Geometry: final body of the model. Coordinates: model frame, mm. A direction names the side the tool comes from. Round coordinates to 2 decimals unless told otherwise and drop trailing zeros. Loops run counter-clockwise (first coordinate to the right, second up) from the corner with the lowest first, then second, coordinate; pieces in that order, holes last. Notation, with made-up numbers: (54.25, 87) -> (67.25, 87) arc R21 ccw to (67.25, 122) -> close; hole circle Ø5 at (-4.5, 36). An arc over 180 degrees is marked (long way). Answer in a Markdown table with one row per item.
```python
from build123d import *

# Parameters (mm, degrees)
SKETCH1_R           = 9
BOSS_EXTRUDE1_DEPTH = 63
SKETCH2_R           = 10
BOSS_EXTRUDE2_DEPTH = 48
SKETCH3_R           = 6
CUT_EXTRUDE1_DEPTH  = 65.567793829
SKETCH4_W           = 1.5
SKETCH4_H           = 27.68
CIRPATTERN1_COUNT   = 4
CHAMFER1_SIZE       = 0.5


with BuildPart() as part:
    # Sketch1 → Boss-Extrude1 (new body)
    with BuildSketch(Plane.XY):
        Circle(SKETCH1_R)
    extrude(amount=BOSS_EXTRUDE1_DEPTH)

    # Sketch2 → Boss-Extrude2 (add)
    with BuildSketch(Plane(origin=(0, 0, 0), x_dir=(-1, 0, 0), z_dir=(0, 0, -1))):
        Circle(SKETCH2_R)
    extrude(amount=-BOSS_EXTRUDE2_DEPTH)

    # Sketch3 → Cut-Extrude1 (cut, through all)
    with BuildSketch(Plane(origin=(0, 0, 0), x_dir=(-1, 0, 0), z_dir=(0, 0, -1))):
        Circle(SKETCH3_R)
    extrude(amount=-CUT_EXTRUDE1_DEPTH, mode=Mode.SUBTRACT)

    # Sketch4 → Cut-Revolve1 (revolve, cut)
    with BuildSketch(Plane(origin=(0, 0, 0), x_dir=(0, 0, -1), z_dir=(1, 0, 0)), mode=Mode.PRIVATE) as cut_revolve1_sk:
        with Locations((-25.75, 0.585439351)):
            Rectangle(SKETCH4_W, SKETCH4_H)
    cut_revolve1 = revolve(cut_revolve1_sk.sketch.rotate(Axis((0, 14.425439351, 26.5), (0, -1, 0)), 180), axis=Axis((0, 14.425439351, 26.5), (0, -1, 0)), mode=Mode.SUBTRACT)

    # CirPattern1: Cut-Revolve1 ×4 about axis
    cirpattern1_axis = Axis((0, 0, 48), (0, 0, -1))
    for i in range(1, CIRPATTERN1_COUNT):
        add(cut_revolve1.rotate(cirpattern1_axis, i * 360 / CIRPATTERN1_COUNT), mode=Mode.SUBTRACT)

    # Chamfer1
    chamfer1_edges = [part.edges().sort_by_distance(p)[0] for p in [
        (6, 0, 63),
    ]]
    chamfer(chamfer1_edges, length=CHAMFER1_SIZE)


solid = part.part
```
Item 1: First-contact query: P1, Ø1.5, axis at y = -5.5, z = 55.5, coming from the +X side; P2, Ø5, axis at x = -1, z = 49.5, coming from the +Y side; P3, Ø1.8, axis at y = 0, z = 26.5, coming from the -X side; P4, Ø2, axis at x = -1.5, z = 55, coming from the -Y side. Flat tips, straight axial feed; report the tip coordinate or a pass-through.
Ans:
| item | result |
|---|---|
| P1 | x = 7.64 |
| P2 | y = 10 |
| P3 | through |
| P4 | y = -8.99 |
Item 2: Section query A-A, the plane y = 0. Output: boundary loops of the cut face in (x, z), and give its area (3 significant figures).
Ans:
| item | result |
|---|---|
| outline | (-10, 0) -> (-6, 0) -> (-6, 25) -> (-10, 25) -> close; (-10, 28) -> (-6, 28) -> (-6, 62.5) -> (-6.5, 63) -> (-9, 63) -> (-9, 48) -> (-10, 48) -> close; (6, 0) -> (10, 0) -> (10, 25) -> (6, 25) -> close; (6, 28) -> (10, 28) -> (10, 48) -> (9, 48) -> (9, 63) -> (6.5, 63) -> (6, 62.5) -> close |
| area | 450 mm2 |
Item 3: Section query C-C, the plane z = 26.5. Output: boundary loops of the cut face in (x, y), and give its area (3 significant figures).
Ans:
| item | result |
|---|---|
| outline | (-9.89, -1.5) arc R10 ccw to (-1.5, -9.89) -> (-1.5, -5.81) arc R6 cw to (-5.81, -1.5) -> close; (-9.89, 1.5) -> (-5.81, 1.5) arc R6 cw to (-1.5, 5.81) -> (-1.5, 9.89) arc R10 ccw to start; (1.5, -9.89) arc R10 ccw to (9.89, -1.5) -> (5.81, -1.5) arc R6 cw to (1.5, -5.81) -> close; (1.5, 5.81) arc R6 cw to (5.81, 1.5) -> (9.89, 1.5) arc R10 ccw to (1.5, 9.89) -> close |
| area | 153 mm2 |
Item 4: Ray query, L1, parallel to X at y = 0, z = 17.5; L2, parallel to Z at x = -8.7, y = 0. Return the intervals inside material, ascending.
Ans:
| item | result |
|---|---|
| L1 | -10 to -6, 6 to 10 |
| L2 | 0 to 25, 28 to 63 |
Item 5: Set-up query: faces 4 (the cylindrical face through (-1.172, 8.923, 55.395)), 5 (the cylindrical face through (-8, 0, 25)). Return all of +Z, -Z, +X, -X, +Y, -Y with unobstructed straight access to the full face (end or side cutting, diameter ignored); none if empty.
Ans:
| item | result |
|---|---|
| face 4 | +Z |
| face 5 | +X, -X |
Item 6: Section query D-D, the plane x = 8. Output: boundary loops of the cut face in (y, z).
Ans:
| item | result |
|---|---|
| outline | (-6, 0) -> (6, 0) -> (6, 48) -> (4.12, 48) -> (4.12, 63) -> (-4.12, 63) -> (-4.12, 48) -> (-6, 48) -> close; hole circle Ø3 at (0, 26.5) |
Item 7: Mould query, pull axis X, two halves, no side actions, for faces 1 (the cylindrical face through (2.17, -9.76, 23.66)), 2 (the cylindrical face through (6, 0, 31)), 3 (the flat face through (3, -6, 63)). Classes: released by +X, released by -X, zero draft, split by the parting line, or undercut.
Ans:
| item | result |
|---|---|
| face 1 | split by the parting line |
| face 2 | undercut |
| face 3 | zero draft |
